Build history of the part. All positions in model axes, mm. Face numbers are marked on the shaded views. A direction names the side the tool comes from. Round coordinates to 2 decimals unless told otherwise and drop trailing zeros. Loops run counter-clockwise (first coordinate to the right, second up) from the corner with the lowest first, then second, coordinate; pieces in that order, holes last. Notation, with made-up numbers: M 79,69 L 112,69 A17 cw 112,86 Z; hole C 65,2.5 d5. An arc over 180 degrees is marked long. Use one line per item in the form item = value. Start each with the question number.
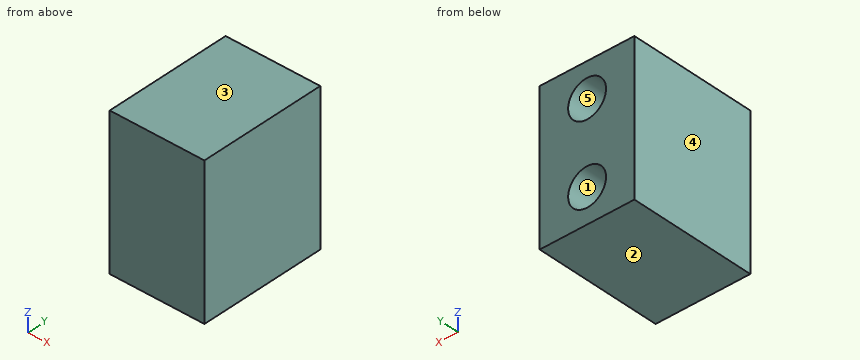
```python
from build123d import *

# Parameters (mm, degrees)
SKETCH2_W              = 80
SKETCH2_H              = 126
BOSS_EXTRUDE1_DEPTH    = 54
M36_TAPPED_HOLE1_D     = 32
M36_TAPPED_HOLE1_DEPTH = 80
M36_TAPPED_HOLE1_TIP   = 9.613769904


with BuildPart() as part:
    # Sketch2 → Boss-Extrude1 (new, symmetric)
    with BuildSketch(Plane(origin=(0, 0, 0), x_dir=(1, 0, 0), z_dir=(0, 1, 0))):
        Rectangle(SKETCH2_W, SKETCH2_H)
    extrude(amount=BOSS_EXTRUDE1_DEPTH, both=True)

    # M36 Tapped Hole1
    with Locations(Plane(origin=(0, 54, 0), x_dir=(1, 0, 0), z_dir=(0, 1, 0))):
        with Locations((0, 34), (0, -34)):
            Hole(M36_TAPPED_HOLE1_D / 2, depth=M36_TAPPED_HOLE1_DEPTH)
            with Locations((0, 0, -(M36_TAPPED_HOLE1_DEPTH + M36_TAPPED_HOLE1_TIP / 2))):  # 118° drill point
                Cone(0, M36_TAPPED_HOLE1_D / 2, M36_TAPPED_HOLE1_TIP, mode=Mode.SUBTRACT)


solid = part.part
```
Q1. Wall check: probe 1 along Z at (x, y) = (0, 16); probe 2 along Z at (x, y) = (5.5, 26); probe 3 along X at (y, z) = (-12, -38.5). Give the ranges that are in metal, low to high.
Q2. Drop a flat-ended pin along its axis: P1, Ø2, axis at x = 0.5, z = 21.5, coming from the +Y side. Give the stop position or say it passes through.
Q3. Saw through at B-B (y = -31). Give the cut face in (x, z).
Q4. Tool access for the marked faces 1 and 2: list every direction of +Z, -Z, +X, -X, +Y, -Y with a clear straight run to the whole face (end or side of a thin tool).
Q5. Saw through at A-A (y = 34.5). Give the cut face in (x, z).
Q6. Pull direction X, two halves, no side cores. Call the marked faces 3, 4 and 5: pulls with the +X half, pulls with the -X half, needs draft (parallel to the pull), parting line crosses it, or undercut.
Filled in:
q1.probe_1 = -63 to -50, -18 to 18, 50 to 63
q1.probe_2 = -63 to -49.02, -18.98 to 18.98, 49.02 to 63
q1.probe_3 = -40 to -15.35, 15.35 to 40
q2.P1 = -27.5
q3.outline = M -40,-63 L 40,-63 L 40,63 L -40,63 Z; hole C 0,-34 d15.36; hole C 0,34 d15.36
q4.face_1 = +Y
q4.face_2 = -Z, +X, -X, +Y, -Y
q5.outline = M -40,-63 L 40,-63 L 40,63 L -40,63 Z; hole C 0,-34 d32; hole C 0,34 d32
q6.face_3 = needs draft
q6.face_4 = pulls with the -X half
q6.face_5 = undercut
